CAD build for the part. Positions are in the model's coordinates, mm. A direction names the side the tool comes from. Give positions to 0.01 mm unless a question says otherwise; leave off trailing zeros. Loops run counter-clockwise (first coordinate to the right, second up) from the corner with the lowest first, then second, coordinate; pieces in that order, holes last.
```python
from build123d import *

# Parameters (mm, degrees)
BOSS_EXTRUDE1_DEPTH = 988
BOSS_EXTRUDE2_START = 70
BOSS_EXTRUDE2_DEPTH = 70
BOSS_EXTRUDE3_DEPTH = 70
CUT_EXTRUDE1_DEPTH  = 70


with BuildPart() as part:
    # Sketch1 → Boss-Extrude1 (new body)
    with BuildSketch(Plane(origin=(574, 0, 0), x_dir=(0, 0, -1), z_dir=(1, 0, 0))):
        with BuildLine():
            Line((40, -28.571428571), (40, 28.571428571))
            ThreePointArc((40, 28.571428571), (36.652648928, 36.652648928), (28.571428571, 40))
            Line((28.571428571, 40), (-28.571428571, 40))
            ThreePointArc((-28.571428571, 40), (-36.652648928, 36.652648928), (-40, 28.571428571))
            Line((-40, 28.571428571), (-40, -28.571428571))
            ThreePointArc((-40, -28.571428571), (-36.652648928, -36.652648928), (-28.571428571, -40))
            Line((-28.571428571, -40), (28.571428571, -40))
            ThreePointArc((28.571428571, -40), (36.652648928, -36.652648928), (40, -28.571428571))
        make_face()
        with BuildLine():
            Line((-34.285714286, -28.571428571), (-34.285714286, 28.571428571))
            ThreePointArc((-34.285714286, 28.571428571), (-32.61203875, 32.61203875), (-28.571428571, 34.285714286))
            Line((-28.571428571, 34.285714286), (28.571428571, 34.285714286))
            ThreePointArc((28.571428571, 34.285714286), (32.61203875, 32.61203875), (34.285714286, 28.571428571))
            Line((34.285714286, 28.571428571), (34.285714286, -28.571428571))
            ThreePointArc((34.285714286, -28.571428571), (32.61203875, -32.61203875), (28.571428571, -34.285714286))
            Line((28.571428571, -34.285714286), (-28.571428571, -34.285714286))
            ThreePointArc((-28.571428571, -34.285714286), (-32.61203875, -32.61203875), (-34.285714286, -28.571428571))
        make_face(mode=Mode.SUBTRACT)
    extrude(amount=-BOSS_EXTRUDE1_DEPTH)

    # Sketch2 → Boss-Extrude2 (add)
    with BuildSketch(Plane(origin=(574, 0, 0), x_dir=(0, 0, -1), z_dir=(1, 0, 0)).offset(BOSS_EXTRUDE2_START)):
        with BuildLine():
            Line((-34.285714286, 28.571428571), (-34.285714286, 38.468861758))
            ThreePointArc((-34.285714286, 38.468861758), (-38.468861758, 34.285714286), (-40, 28.571428571))
            Line((-40, 28.571428571), (-40, -28.571428571))
            ThreePointArc((-40, -28.571428571), (-38.468861758, -34.285714286), (-34.285714286, -38.468861758))
            Line((-34.285714286, -38.468861758), (-34.285714286, -28.571428571))
            Line((-34.285714286, -28.571428571), (-34.285714286, 28.571428571))
        make_face()
    extrude(amount=-BOSS_EXTRUDE2_DEPTH)

    # Sketch3 → Boss-Extrude3 (add)
    with BuildSketch(Plane.ZY.offset(414)):
        with BuildLine():
            Line((34.285714286, -28.571428571), (34.285714286, -38.468861758))
            ThreePointArc((34.285714286, -38.468861758), (38.468861758, -34.285714286), (40, -28.571428571))
            Line((40, -28.571428571), (40, 28.571428571))
            ThreePointArc((40, 28.571428571), (38.468861758, 34.285714286), (34.285714286, 38.468861758))
            Line((34.285714286, 38.468861758), (34.285714286, -28.571428571))
        make_face()
    extrude(amount=BOSS_EXTRUDE3_DEPTH)

    # Sketch4 → Cut-Extrude1 (cut)
    with BuildSketch(Plane.XY.offset(40)):
        with BuildLine():
            Line((-464, 24.25), (-444, 24.25))
            ThreePointArc((-444, 24.25), (-439.75, 20), (-444, 15.75))
            Line((-444, 15.75), (-464, 15.75))
            ThreePointArc((-464, 15.75), (-468.25, 20), (-464, 24.25))
        make_face()
        with BuildLine():
            Line((-464, -24.25), (-444, -24.25))
            ThreePointArc((-444, -24.25), (-439.75, -20), (-444, -15.75))
            Line((-444, -15.75), (-464, -15.75))
            ThreePointArc((-464, -15.75), (-468.25, -20), (-464, -24.25))
        make_face()
        with BuildLine():
            Line((604, 24.25), (624, 24.25))
            ThreePointArc((624, 24.25), (628.25, 20), (624, 15.75))
            Line((624, 15.75), (604, 15.75))
            ThreePointArc((604, 15.75), (599.75, 20), (604, 24.25))
        make_face()
        with BuildLine():
            Line((604, -24.25), (624, -24.25))
            ThreePointArc((624, -24.25), (628.25, -20), (624, -15.75))
            Line((624, -15.75), (604, -15.75))
            ThreePointArc((604, -15.75), (599.75, -20), (604, -24.25))
        make_face()
    extrude(amount=-CUT_EXTRUDE1_DEPTH, mode=Mode.SUBTRACT)


solid = part.part
```
1. Drop flat-ended pins along their axis: pin 1 (4.5 mm diameter, centred on x = -455, z = 36, fed in from -Y); pin 2 (1.7 mm diameter, centred on x = -450.5, z = 37.5, fed in from +Y); pin 3 (3 mm diameter, centred on x = 616, z = 36.5, fed in from +Y). Give the stop position or say it passes through.
Responses:
pin 1: stops at y = -38.47
pin 2: stops at y = 36.66
pin 3: stops at y = 38.02
2. Saw through at A-A, the plane y = 1. List the corners of the cut face in (x, z), and give its area (3 significant figures).
Responses:
outline: (-484, 34.29) - (644, 34.29) - (644, 40) - (-484, 40) - close; (-414, -40) - (574, -40) - (574, -34.29) - (-414, -34.29) - close
area: 12,100 mm2
3. Pull direction Y, two halves, no side cores. Call faces 1 (the face through (87, 40, 0)), 2 (the face through (87, 0, -34.286)), 3 (the face through (574, -3, -36)), 4 (the face through (87, 34.286, 0)): released by +Y, released by -Y, zero draft, split by the parting line, or undercut.
Responses:
face 1: released by +Y
face 2: undercut
face 3: zero draft
face 4: undercut
4. Probe line 1 along Z through (x, y) = (15.5, -26); line 2 along Y through (x, z) = (479, -34.5). List the from-to ranges inside material, lowest first.
Responses:
line 1: z = -40 to -34.29, 34.29 to 40
line 2: y = -38.34 to 38.34
5. Tool access for faces 5 (the face through (87, -34.286, 0)), 6 (the face through (-414, -3, -36)), 7 (the face through (87, -40, 0)): list every direction of +Z, -Z, +X, -X, +Y, -Y with a clear straight run to the whole face (end or side of a thin tool).
Responses:
face 5: +X, -X
face 6: -Z, -X, +Y, -Y
face 7: +Z, -Z, +X, -X, -Y
6. Saw through at B-B, the plane x = 533. List the corners of the cut face in (y, z).
Responses:
outline: (-40, -28.57) arc R11.43 ccw to (-28.57, -40) - (28.57, -40) arc R11.43 ccw to (40, -28.57) - (40, 28.57) arc R11.43 ccw to (28.57, 40) - (-28.57, 40) arc R11.43 ccw to (-40, 28.57) - close; hole (-34.29, -28.57) arc R5.71 ccw to (-28.57, -34.29) - (28.57, -34.29) arc R5.71 ccw to (34.29, -28.57) - (34.29, 28.57) arc R5.71 ccw to (28.57, 34.29) - (-28.57, 34.29) arc R5.71 ccw to (-34.29, 28.57) - close
